from build123d import *

# Parameters (mm, degrees)
SKETCH1_W            = 200
SKETCH1_H            = 200
BOSS_EXTRUDE1_DEPTH  = 5
SKETCH2_R            = 7.5
CUT_EXTRUDE1_DEPTH   = 10
LPATTERN1_COUNT      = 2
LPATTERN1_PITCH      = 180
LPATTERN1_COUNT_DIR2 = 3
LPATTERN1_PITCH_DIR2 = 80


with BuildPart() as part:
    # Sketch1 → Boss-Extrude1 (new, symmetric)
    with BuildSketch(Plane(origin=(0, 0, 0), x_dir=(1, 0, 0), z_dir=(0, 1, 0))):
        Rectangle(SKETCH1_W, SKETCH1_H)
    extrude(amount=BOSS_EXTRUDE1_DEPTH, both=True)

    # Sketch2 → Cut-Extrude1 (cut)
    with BuildSketch(Plane(origin=(0, 5, 0), x_dir=(1, 0, 0), z_dir=(0, 1, 0))):
        with Locations(Location((80, 90, 0), (0, 0, 270))):
            Circle(SKETCH2_R)
    cut_extrude1 = extrude(amount=-CUT_EXTRUDE1_DEPTH, mode=Mode.SUBTRACT)

    # LPattern1: Cut-Extrude1 2 × 3
    with Locations(*[(-j * LPATTERN1_PITCH_DIR2, 0, i * LPATTERN1_PITCH) for i in range(LPATTERN1_COUNT) for j in range(LPATTERN1_COUNT_DIR2) if (i, j) != (0, 0)]):
        add(cut_extrude1, mode=Mode.SUBTRACT)


solid = part.part
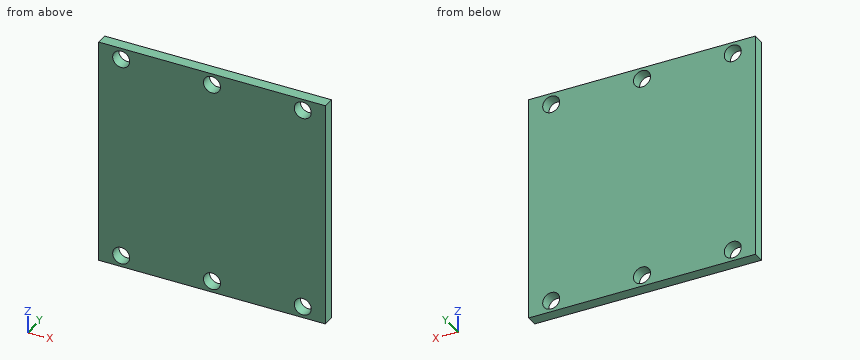
Geometry check sheet. Reference: the model listing, model coordinates, mm. Give positions to 0.01 mm unless a question says otherwise; leave off trailing zeros. Loops run counter-clockwise (first coordinate to the right, second up) from the corner with the lowest first, then second, coordinate; pieces in that order, holes last. Notation, with made-up numbers: M 30.25,10 L 72.25,10 A22 ccw 72.25,17 Z; hole C 51,22 d4. An arc over 180 degrees is marked long. Answer as a JSON object with one key per item and string values. Group by question number.
Item 1: Sectioned sample at D-D on x = -5. Record the boundary of the cut face in (y, z), plus the area to 3 significant figures.
Item 2: Sectioned sample at C-C on z = 90. Record the boundary of the cut face in (x, y).
Item 3: Sectioned sample at A-A on x = 80. Record the boundary of the cut face in (y, z).
Item 4: Sectioned sample at B-B on y = 2.5. Record the boundary of the cut face in (x, z).
Item 5: Material ranges on L1, parallel to X at y = 2.5, z = -90; L2, parallel to Z at x = 81, y = -1, recorded low to high.
Findings below:
{
 "1": {"outline": "M -5,-100 L 5,-100 L 5,-95.59 L -5,-95.59 Z; M -5,-84.41 L 5,-84.41 L 5,84.41 L -5,84.41 Z; M -5,95.59 L 5,95.59 L 5,100 L -5,100 Z", "area": "1,780 mm2"},
 "2": {"outline": "M -100,-5 L -87.5,-5 L -87.5,5 L -100,5 Z; M -72.5,-5 L -7.5,-5 L -7.5,5 L -72.5,5 Z; M 7.5,-5 L 72.5,-5 L 72.5,5 L 7.5,5 Z; M 87.5,-5 L 100,-5 L 100,5 L 87.5,5 Z"},
 "3": {"outline": "M -5,-100 L 5,-100 L 5,-97.5 L -5,-97.5 Z; M -5,-82.5 L 5,-82.5 L 5,82.5 L -5,82.5 Z; M -5,97.5 L 5,97.5 L 5,100 L -5,100 Z"},
 "4": {"outline": "M -100,-100 L 100,-100 L 100,100 L -100,100 Z; hole C -80,-90 d15; hole C -80,90 d15; hole C 0,-90 d15; hole C 0,90 d15; hole C 80,-90 d15; hole C 80,90 d15"},
 "5": {"L1": "-100 to -87.5, -72.5 to -7.5, 7.5 to 72.5, 87.5 to 100", "L2": "-100 to -97.43, -82.57 to 82.57, 97.43 to 100"}
}
